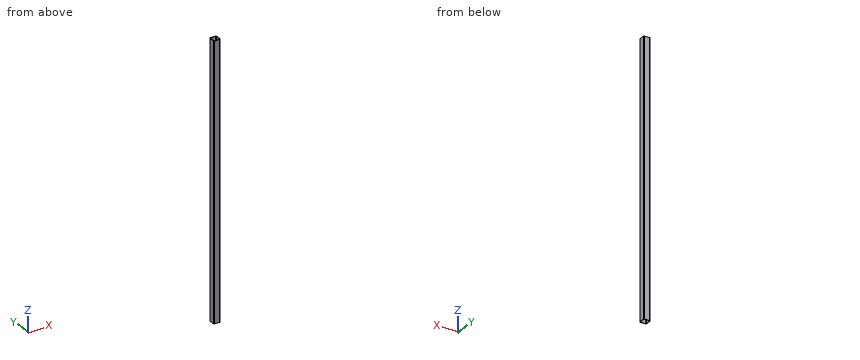
```python
from build123d import *

# Parameters (mm, degrees)
GB_6728_1986_050_X_50_X_3_1_DEPTH = 2070


with BuildPart() as part:
    # Sketch1 → Gb／6728-1986方形空心型钢 050 X 50 X 3(1) (new body)
    with BuildSketch(Plane.YX.offset(-1035)):
        with BuildLine():
            Line((-19, -25), (19, -25))
            ThreePointArc((19, -25), (23.242640687, -23.242640687), (25, -19))
            Line((25, -19), (25, 19))
            ThreePointArc((25, 19), (23.242640687, 23.242640687), (19, 25))
            Line((19, 25), (-19, 25))
            ThreePointArc((-19, 25), (-23.242640687, 23.242640687), (-25, 19))
            Line((-25, 19), (-25, -19))
            ThreePointArc((-25, -19), (-23.242640687, -23.242640687), (-19, -25))
        make_face()
        with BuildLine():
            Line((-19, -22), (19, -22))
            ThreePointArc((19, -22), (21.121320344, -21.121320344), (22, -19))
            Line((22, -19), (22, 19))
            ThreePointArc((22, 19), (21.121320344, 21.121320344), (19, 22))
            Line((19, 22), (-19, 22))
            ThreePointArc((-19, 22), (-21.121320344, 21.121320344), (-22, 19))
            Line((-22, 19), (-22, -19))
            ThreePointArc((-22, -19), (-21.121320344, -21.121320344), (-19, -22))
        make_face(mode=Mode.SUBTRACT)
    extrude(amount=GB_6728_1986_050_X_50_X_3_1_DEPTH)


solid = part.part
```
Work out the finished part from the listing and answer in its coordinate system (mm). Give positions to 0.01 mm unless a question says otherwise; leave off trailing zeros. Order: outer loops, then holes, each group sorted by start corner. A loop starts at its lowest first (then second) coordinate and runs counter-clockwise, first axis right, second up. Notation, with made-up numbers: M -6.5,16 L 25.5,16 A17 cw 25.5,34 Z; hole C 23.25,-24 d11. An arc over 180 degrees is marked long. Return JSON: item names as keys, results as strings.
1) Section A-A, the plane y = 11 is taken. Write down the section's boundary in (x, z), plus the area to 3 significant figures.
Resolved:
{"outline": "M -25,-1035 L -22,-1035 L -22,1035 L -25,1035 Z; M 22,-1035 L 25,-1035 L 25,1035 L 22,1035 Z", "area": "12,400 mm^2"}
2) Straight lines are drawn through the part: line 1 along X through (y, z) = (-11.5, 822); line 2 along X through (y, z) = (20, 623.5). For each, find the intervals that lie inside material, in ascending order. Write a range as [from, to].
Resolved:
{"line 1": "[-25, -22], [22, 25]", "line 2": "[-24.92, -21.83], [21.83, 24.92]"}
3) Section B-B, the plane z = 382 is taken. Write down the section's boundary in (x, y), plus the area to 3 significant figures.
Resolved:
{"outline": "M -25,-19 A6 ccw -19,-25 L 19,-25 A6 ccw 25,-19 L 25,19 A6 ccw 19,25 L -19,25 A6 ccw -25,19 Z; hole M -22,-19 A3 ccw -19,-22 L 19,-22 A3 ccw 22,-19 L 22,19 A3 ccw 19,22 L -19,22 A3 ccw -22,19 Z", "area": "541 mm^2"}
